Drawing for the job (mm, zero at the part's lowest x, y, z). A direction names the side the tool comes from. Coordinates: 2 decimals unless noted, no trailing zeros. Order: outer loops, then holes, each group sorted by start corner. A loop starts at its lowest first (then second) coordinate and runs counter-clockwise, first axis right, second up.
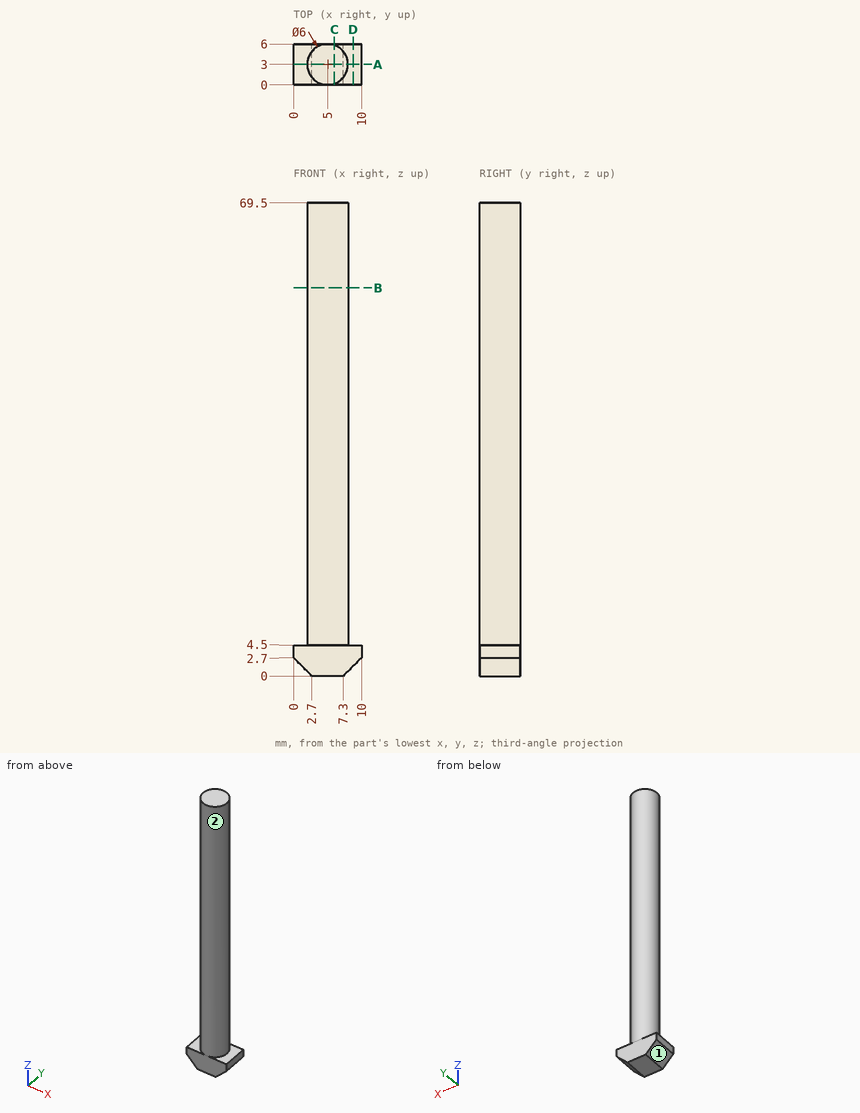
(1) Probe line 1 (Z direction, x = 7, y = 5.75); line 2 (X direction, y = 5.15, z = 10); line 3 (Z direction, x = 7.5, y = 1.7). List the from-to ranges inside material, lowest first.
(2) Tool access for the marked faces 1 and 2: list every direction of +Z, -Z, +X, -X, +Y, -Y with a clear straight run to the whole face (end or side of a thin tool).
(3) Slice it at D-D, the plane x = 8.75. Give the cut face in (y, z).
(4) Slice it at A-A, the plane y = 3. Give the cut face in (x, z), then the cut area to 3 significant figures.
(5) Slice it at B-B, the plane z = 57. Give the cut face in (x, y).
(6) Slice it at C-C, the plane x = 6. Give the cut face in (y, z).
(7) Drop flat-ended pins along their axis: pin 1 (3 mm diameter, centred on x = 7, z = 32, fed in from +Y); pin 2 (1 mm diameter, centred on y = 3, z = 53, fed in from +X); pin 3 (2 mm diameter, centred on x = 8, z = 42.5, fed in from +Y). Give the stop position or say it passes through.
Here are the results:
1. line 1: z = 0 to 4.5
1. line 2: x = 2.91 to 7.09
1. line 3: z = 0.2 to 69.5
2. face 1: -Z, -X, +Y, -Y
2. face 2: +Z
3. outline: (0, 1.45) - (6, 1.45) - (6, 4.5) - (0, 4.5) - close
4. outline: (0, 2.7) - (2.7, 0) - (7.3, 0) - (10, 2.7) - (10, 4.5) - (8, 4.5) - (8, 69.5) - (2, 69.5) - (2, 4.5) - (0, 4.5) - close
4. area: 428 mm2
5. outline: circle Ø6 at (5, 3)
6. outline: (0, 0) - (6, 0) - (6, 4.5) - (5.83, 4.5) - (5.83, 69.5) - (0.17, 69.5) - (0.17, 4.5) - (0, 4.5) - close
7. pin 1: stops at y = 5.96
7. pin 2: stops at x = 8
7. pin 3: stops at y = 5.24
